Can you work these out from the model? Positions are in its coordinate system, mm. A direction names the side the tool comes from. Give positions to 0.01 mm unless a question says otherwise; leave off trailing zeros. Write each loop counter-clockwise with the first axis right and the second up, starting at its lowest first coordinate (ties: lowest second). Pieces come first, ordered by that corner, then holes.
```python
from build123d import *

# Parameters (mm, degrees)
EXTRUDE_1_DEPTH = 1165
EXTRUDE_START   = -110
EXTRUDE_2_DEPTH = 10
EXTRUDE_4_REACH = 1205.598
SKETCH_4_W      = 256
SKETCH_4_H      = 10


with BuildPart() as part:
    # 草图1 → 凸台-拉伸1 (new body)
    with BuildSketch(Plane.XY):
        with BuildLine():
            Line((-110, 140), (110, 140))
            ThreePointArc((110, 140), (131.213203436, 131.213203436), (140, 110))
            Line((140, 110), (140, -110))
            ThreePointArc((140, -110), (131.213203436, -131.213203436), (110, -140))
            Line((110, -140), (-110, -140))
            ThreePointArc((-110, -140), (-131.213203436, -131.213203436), (-140, -110))
            Line((-140, -110), (-140, 110))
            ThreePointArc((-140, 110), (-131.213203436, 131.213203436), (-110, 140))
        make_face()
        with BuildLine():
            Line((-110, 128), (110, 128))
            ThreePointArc((110, 128), (122.727922061, 122.727922061), (128, 110))
            Line((128, 110), (128, -110))
            ThreePointArc((128, -110), (122.727922061, -122.727922061), (110, -128))
            Line((110, -128), (-110, -128))
            ThreePointArc((-110, -128), (-122.727922061, -122.727922061), (-128, -110))
            Line((-128, -110), (-128, 110))
            ThreePointArc((-128, 110), (-122.727922061, 122.727922061), (-110, 128))
        make_face(mode=Mode.SUBTRACT)
    extrude(amount=EXTRUDE_1_DEPTH)

    # 草图2 → 凸台-拉伸2 (add)
    with BuildSketch(Plane.XY.offset(1165).offset(EXTRUDE_START)):
        with BuildLine():
            Line((128, -110), (128, 110))
            ThreePointArc((128, 110), (122.727922061, 122.727922061), (110, 128))
            Line((110, 128), (-110, 128))
            ThreePointArc((-110, 128), (-122.727922061, 122.727922061), (-128, 110))
            Line((-128, 110), (-128, -110))
            ThreePointArc((-128, -110), (-122.727922061, -122.727922061), (-110, -128))
            Line((-110, -128), (110, -128))
            ThreePointArc((110, -128), (122.727922061, -122.727922061), (128, -110))
        make_face()
    extrude_2 = extrude(amount=EXTRUDE_2_DEPTH)

    # 镜向1: 凸台-拉伸2 across plane
    add(extrude_2.mirror(Plane.XY.offset(582.5)))

    # 凸台-拉伸4: up to this face of the body (flat: up to its plane)
    extrude_4_end = Plane(part.part.faces().sort_by_distance((0, 128, 50))[0])
    # 草图4 → 凸台-拉伸4 (add, up to the picked face)
    with BuildSketch(Plane(origin=(0, -128, 0), x_dir=(1, 0, 0), z_dir=(0, 1, 0)), mode=Mode.PRIVATE) as extrude_4_sk1:
        with Locations((0, -740)):
            Rectangle(SKETCH_4_W, SKETCH_4_H)
    extrude_4_tool1 = split(extrude(extrude_4_sk1.sketch, amount=EXTRUDE_4_REACH, mode=Mode.PRIVATE), bisect_by=extrude_4_end, keep=Keep.BOTH, mode=Mode.PRIVATE)
    # 草图4 → 凸台-拉伸4 (add, up to the picked face)
    with BuildSketch(Plane(origin=(0, -128, 0), x_dir=(1, 0, 0), z_dir=(0, 1, 0)), mode=Mode.PRIVATE) as extrude_4_sk2:
        with Locations((0, -425)):
            Rectangle(SKETCH_4_W, SKETCH_4_H)
    extrude_4_tool2 = split(extrude(extrude_4_sk2.sketch, amount=EXTRUDE_4_REACH, mode=Mode.PRIVATE), bisect_by=extrude_4_end, keep=Keep.BOTH, mode=Mode.PRIVATE)
    add(extrude_4_tool1.solids().sort_by(Axis((0, -128, 740), (0, 1, 0)))[0])
    add(extrude_4_tool2.solids().sort_by(Axis((0, -128, 425), (0, 1, 0)))[0])


solid = part.part
```
1) Suppose I cut it at B-B on z = 784.5. Write out the boundary of the cut face in (x, y), plus the area to 3 significant figures.
Values follow:
outline: (-140, -110) arc R30 ccw to (-110, -140) - (110, -140) arc R30 ccw to (140, -110) - (140, 110) arc R30 ccw to (110, 140) - (-110, 140) arc R30 ccw to (-140, 110) - close; hole (-128, -110) arc R18 ccw to (-110, -128) - (110, -128) arc R18 ccw to (128, -110) - (128, 110) arc R18 ccw to (110, 128) - (-110, 128) arc R18 ccw to (-128, 110) - close
area: 12,400 mm2
2) If we mould it in two halves opening along X, with no side actions, what happens to faces 4 (the face through (-131.445, 130.979, 574.345)), 5 (the face through (-128, -2, 263)), 6 (the face through (-2, 140, 574)), 7 (the face through (131.445, -130.979, 574.345))? For each: +X half, -X half, draft (parallel to the pull), parting line (faces both ways), or undercut.
Values follow:
face 4: -X half
face 5: undercut
face 6: draft
face 7: +X half
3) Suppose I cut it at A-A on y = -22. Write out the boundary of the cut face in (x, z).
Values follow:
outline: (-140, 0) - (-128, 0) - (-128, 100) - (128, 100) - (128, 0) - (140, 0) - (140, 1165) - (128, 1165) - (128, 1065) - (-128, 1065) - (-128, 1165) - (-140, 1165) - close; hole (-128, 110) - (128, 110) - (128, 420) - (-128, 420) - close; hole (-128, 430) - (128, 430) - (128, 735) - (-128, 735) - close; hole (-128, 745) - (128, 745) - (128, 1055) - (-128, 1055) - close
4) Please list where these lines run through material, in increasing order: L1, parallel to Z at x = 124, y = -74; L2, parallel to X at y = -4, z = 226.5.
Values follow:
L1: z = 100 to 110, 420 to 430, 735 to 745, 1055 to 1065
L2: x = -140 to -128, 128 to 140
5) For pin 1 Ø1 at (x, y) = (15, 7.5) entering from -Z, with a flat end and sliding along its axis, tell me the tip position at first contact or that it passes through.
Values follow:
pin 1: stops at z = 100
6) For faces 1 (the face through (128, 2, 263)), 2 (the face through (128, 2, 1114)), 3 (the face through (-128, -2, 49)), which set-ups out of +Z, -Z, +X, -X, +Y, -Y let a thin tool reach every point of the face, with its end or its side?
Values follow:
face 1: none
face 2: +Z
face 3: -Z
